Can you work these out from the model? Positions are in its coordinate system, mm. A direction names the side the tool comes from. Give positions to 0.01 mm unless a question says otherwise; leave off trailing zeros. Loops run counter-clockwise (first coordinate to the right, second up) from the corner with the lowest first, then second, coordinate; pieces in that order, holes last. Notation, with made-up numbers: M 38.25,36.5 L 86.25,36.5 A22 ccw 86.25,62.5 Z; hole C 17.25,46.25 d9. An arc over 180 degrees is marked long. Put each result on its own line as item: value. Start each with the question number.
1) Imagine slicing it at A-A (y = 20.75). Write out the boundary of the cut face in (x, z), then the cut area to 3 significant figures.
2) Imagine slicing it at B-B (z = 32). Write out the boundary of the cut face in (x, y), then the cut area to 3 significant figures.
3) Please list where these lines run through material, in increasing order: line 1 along X through (y, z) = (20.25, 30); line 2 along Y through (x, z) = (13.5, 23.5). Write a range as from..to.
4) For P1, Ø12, axis at x = 29.5, z = 41, coming from the +Y side; P2, Ø13.5, axis at y = 15, z = 118, coming from the -X side, each with a flat end and sliding along its axis, tell me the tip position at first contact or that it passes through.
5) If we mould it in two halves opening along Z, with no side actions, what happens to faces 1 (the flat face through (23.3, 2.8, 0)), 2 (the flat face through (47, 16, 84)), 3 (the flat face through (26.7, 2.8, 170))? For each: +Z half, -Z half, draft (parallel to the pull), parting line (faces both ways), or undercut.
6) For faces 4 (the flat face through (25, 3, 84)), 5 (the flat face through (50, 15, 84)), which set-ups out of +Z, -Z, +X, -X, +Y, -Y let a thin tool reach every point of the face, with its end or its side?
7) Imagine slicing it at C-C (x = 12). Write out the boundary of the cut face in (y, z), then the cut area to 3 significant figures.
from build123d import *

# Parameters (mm, degrees)
EXTRUDE_1_DEPTH     = 340
CUT_EXTRUDE_1_DEPTH = 170


with BuildPart() as part:
    # 草图1 → 凸台-拉伸1 (new body)
    with BuildSketch(Plane.XY):
        Polygon((0, 0), (0, 30), (3, 30), (3, 3), (47, 3), (47, 30), (50, 30), (50, 0), align=None)
    extrude(amount=EXTRUDE_1_DEPTH)

    # 草图2 → 切除-拉伸1 (cut)
    with BuildSketch(Plane.XY.offset(340)):
        Polygon((0, 0), (50, 0), (50, 30), (47, 30), (47, 3), (3, 3), (3, 30), (0, 30), align=None)
    extrude(amount=-CUT_EXTRUDE_1_DEPTH, mode=Mode.SUBTRACT)


solid = part.part
Recorded:
1. outline: M 0,0 L 3,0 L 3,170 L 0,170 Z; M 47,0 L 50,0 L 50,170 L 47,170 Z
1. area: 1,020 mm²
2. outline: M 0,0 L 50,0 L 50,30 L 47,30 L 47,3 L 3,3 L 3,30 L 0,30 Z
2. area: 312 mm²
3. line 1: 0..3, 47..50
3. line 2: 0..3
4. P1: y = 3
4. P2: x = 0
5. face 1: -Z half
5. face 2: draft
5. face 3: +Z half
6. face 4: +Z, -Z, +Y
6. face 5: +Z, -Z, +X, +Y, -Y
7. outline: M 0,0 L 3,0 L 3,170 L 0,170 Z
7. area: 510 mm²
